from build123d import *

# Parameters (mm, degrees)
BOSS_EXTRUDE1_DEPTH = 80
CUT_EXTRUDE1_DEPTH  = 15
CUT_EXTRUDE2_DEPTH  = 32
M20_TAPPED_HOLE1_D  = 17.5
HOLE1_D             = 8.4
HOLE1_CBORE_D       = 15
HOLE1_CBORE_DEPTH   = 20
CHAMFER1_SIZE       = 2


with BuildPart() as part:
    # Sketch2 → Boss-Extrude1 (new body)
    with BuildSketch(Plane.XY):
        Polygon((-36.962834249, 9.808501666), (-36.962834249, -38.191498334), (20.037165751, -38.191498334), (20.037165751, -30.191498334), (48.037165751, -30.191498334), (48.037165751, 9.808501666), align=None)
    extrude(amount=BOSS_EXTRUDE1_DEPTH)

    # Sketch3 → Cut-Extrude1 (cut)
    with BuildSketch(Plane.XY.offset(80)):
        with BuildLine():
            Line((-19.462834249, -9.191498334), (-19.462834249, 9.808501666))
            Line((-19.462834249, 9.808501666), (5.537165751, 9.808501666))
            Line((5.537165751, 9.808501666), (5.537165751, -9.191498334))
            ThreePointArc((5.537165751, -9.191498334), (-6.962834249, -21.691498334), (-19.462834249, -9.191498334))
        make_face()
    extrude(amount=-CUT_EXTRUDE1_DEPTH, mode=Mode.SUBTRACT)

    # Sketch4 → Cut-Extrude2 (cut)
    with BuildSketch(Plane.XY.offset(65)):
        with BuildLine():
            Line((-25.962834249, -9.191498334), (-25.962834249, 9.808501666))
            Line((-25.962834249, 9.808501666), (12.037165751, 9.808501666))
            Line((12.037165751, 9.808501666), (12.037165751, -9.191498334))
            ThreePointArc((12.037165751, -9.191498334), (-6.962834249, -28.191498334), (-25.962834249, -9.191498334))
        make_face()
    extrude(amount=-CUT_EXTRUDE2_DEPTH, mode=Mode.SUBTRACT)

    # M20 Tapped Hole1 (through all)
    with Locations(Plane.XY.offset(33)):
        with Locations((-6.962834249, -9.191498334)):
            Hole(M20_TAPPED_HOLE1_D / 2)

    # Hole1 (through all)
    with Locations(Plane(origin=(0, 9.808501666, 0), x_dir=(1, 0, 0), z_dir=(0, 1, 0))):
        with Locations((36.037165751, -10), (36.037165751, -40), (36.037165751, -70)):
            CounterBoreHole(HOLE1_D / 2, HOLE1_CBORE_D / 2, HOLE1_CBORE_DEPTH)

    # Chamfer1
    chamfer1_edges = [part.edges().sort_by_distance(p)[0] for p in [
        (-19.462834249, 9.808501666, 72.5),
        (48.037165751, -10.191498334, 80),
        (5.537165751, 9.808501666, 72.5),
        (48.037165751, -10.191498334, 0),
        (-36.962834249, -14.191498334, 0),
        (-36.962834249, -14.191498334, 80),
    ]]
    chamfer(chamfer1_edges, length=CHAMFER1_SIZE)


solid = part.part
Source: CAD feature listing. Evaluate the final solid. Frame: model axes, mm. A direction names the side the tool comes from. Give positions to 0.01 mm unless a question says otherwise; leave off trailing zeros. Order: outer loops, then holes, each group sorted by start corner. A loop starts at its lowest first (then second) coordinate and runs counter-clockwise, first axis right, second up. Notation, with made-up numbers: (36, -20) -> (59, -20) arc R20 cw to (59, 17) -> close; hole circle Ø7 at (2.5, 82.25). An arc over 180 degrees is marked (long way). Use a Markdown table: item, result.
1) Ray query, line 1 along X through (y, z) = (-1.5, 69.5); line 2 along Z through (x, y) = (0, -26); line 3 along Z through (x, y) = (34, -7.5). Return the intervals inside material, ascending. Write a range as [from, to].
Answer list:
| item | result |
|---|---|
| line 1 | [-36.96, -19.46], [5.54, 28.55], [43.52, 48.04] |
| line 2 | [0, 33], [65, 80] |
| line 3 | [0, 2.78], [17.22, 32.78], [47.22, 62.78], [77.22, 80] |
2) Contact query for flat-ended pins moving along their axis: P1, Ø4, axis at x = -1.5, y = -19.5, coming from the -Z side; P2, Ø13.5, axis at x = 36.04, z = 70, coming from the +Y side; P3, Ø5, axis at x = -5, z = 65.5, coming from the +Y side; P4, Ø12, axis at x = 36.04, z = 70, coming from the -Y side. Output: stop coordinate, or through.
Answer list:
| item | result |
|---|---|
| P1 | z = 0 |
| P2 | y = -10.19 |
| P3 | y = -20.87 |
| P4 | y = -30.19 |
3) Section query D-D, the plane x = 35. Return the cut outline in (y, z).
Answer list:
| item | result |
|---|---|
| outline | (-30.19, 0) -> (9.81, 0) -> (9.81, 2.57) -> (-10.19, 2.57) -> (-10.19, 5.93) -> (-30.19, 5.93) -> close; (-30.19, 14.07) -> (-10.19, 14.07) -> (-10.19, 17.43) -> (9.81, 17.43) -> (9.81, 32.57) -> (-10.19, 32.57) -> (-10.19, 35.93) -> (-30.19, 35.93) -> close; (-30.19, 44.07) -> (-10.19, 44.07) -> (-10.19, 47.43) -> (9.81, 47.43) -> (9.81, 62.57) -> (-10.19, 62.57) -> (-10.19, 65.93) -> (-30.19, 65.93) -> close; (-30.19, 74.07) -> (-10.19, 74.07) -> (-10.19, 77.43) -> (9.81, 77.43) -> (9.81, 80) -> (-30.19, 80) -> close |
4) Reachability of faces 1 (the flat face through (-2, -22, 65)), 2 (the flat face through (20.037, -34, 39)), 3 (the flat face through (6.52, 8.79, 72.6)), 4 (the flat face through (47.051, -10.471, 1.014)), 5 (the cylindrical face through (34.099, -20.331, 73.726)) from +Z, -Z, +X, -X, +Y, -Y: full face, straight path, thin tool, end or side. Return the list, or none.
Answer list:
| item | result |
|---|---|
| face 1 | +Y |
| face 2 | +Z, -Z, +X, -Y |
| face 3 | +Z, +Y |
| face 4 | -Z, +X, +Y, -Y |
| face 5 | +Y, -Y |
5) Section query C-C, the plane z = 10. Return the cut outline in (x, y), then the cut area to 3 significant figures.
Answer list:
| item | result |
|---|---|
| outline | (-36.96, -38.19) -> (20.04, -38.19) -> (20.04, -30.19) -> (31.84, -30.19) -> (31.84, -10.19) -> (28.54, -10.19) -> (28.54, 9.81) -> (-36.96, 9.81) -> close; (40.24, -30.19) -> (48.04, -30.19) -> (48.04, 9.81) -> (43.54, 9.81) -> (43.54, -10.19) -> (40.24, -10.19) -> close; hole circle Ø17.5 at (-6.96, -9.19) |
| area | 3,150 mm² |
6) Mould query, pull axis Z, two halves, no side actions, for faces 6 (the cylindrical face through (33.78, -20.33, 36.46)), 7 (the flat face through (-19.463, -1, 73)), 8 (the flat face through (5, -14, 80)). Classes: +Z half, -Z half, draft (parallel to the pull), parting line (faces both ways), or undercut.
Answer list:
| item | result |
|---|---|
| face 6 | undercut |
| face 7 | draft |
| face 8 | +Z half |
7) Section query A-A, the plane z = 40. Return the cut outline in (x, y).
Answer list:
| item | result |
|---|---|
| outline | (-36.96, -38.19) -> (20.04, -38.19) -> (20.04, -30.19) -> (31.84, -30.19) -> (31.84, -10.19) -> (28.54, -10.19) -> (28.54, 9.81) -> (12.04, 9.81) -> (12.04, -9.19) arc R19 cw to (-25.96, -9.19) -> (-25.96, 9.81) -> (-36.96, 9.81) -> close; (40.24, -30.19) -> (48.04, -30.19) -> (48.04, 9.81) -> (43.54, 9.81) -> (43.54, -10.19) -> (40.24, -10.19) -> close |
8) Section query B-B, the plane y = -3. Return the cut outline in (x, z).
Answer list:
| item | result |
|---|---|
| outline | (-36.96, 2) -> (-34.96, 0) -> (-13.15, 0) -> (-13.15, 33) -> (-25.96, 33) -> (-25.96, 65) -> (-19.46, 65) -> (-19.46, 80) -> (-34.96, 80) -> (-36.96, 78) -> close; (-0.78, 0) -> (46.04, 0) -> (48.04, 2) -> (48.04, 78) -> (46.04, 80) -> (5.54, 80) -> (5.54, 65) -> (12.04, 65) -> (12.04, 33) -> (-0.78, 33) -> close; hole circle Ø15 at (36.04, 10); hole circle Ø15 at (36.04, 40); hole circle Ø15 at (36.04, 70) |
